Input: part model. Units: mm. Frame: model coordinates. A direction names the side the tool comes from. Give positions to 0.01 mm unless a question says otherwise; leave off trailing zeros. Loops run counter-clockwise (first coordinate to the right, second up) from the corner with the lowest first, then second, coordinate; pieces in that order, holes last.
from build123d import *

# Parameters (mm, degrees)
BOSS_EXTRUDE1_DEPTH     = 235
CUT_EXTRUDE1_DEPTH      = 252.322501977
CUT_EXTRUDE1_DEPTH_BACK = 252.322501977
SKETCH_1_R              = 16


with BuildPart() as part:
    # Sketch1 → Boss-Extrude1 (new, symmetric)
    with BuildSketch(Plane.XY):
        with BuildLine():
            Line((-53, -63), (53, -63))
            ThreePointArc((53, -63), (60.071067812, -60.071067812), (63, -53))
            Line((63, -53), (63, 53))
            ThreePointArc((63, 53), (60.071067812, 60.071067812), (53, 63))
            Line((53, 63), (-53, 63))
            ThreePointArc((-53, 63), (-60.071067812, 60.071067812), (-63, 53))
            Line((-63, 53), (-63, -53))
            ThreePointArc((-63, -53), (-60.071067812, -60.071067812), (-53, -63))
        make_face()
        with BuildLine():
            Line((-53, -58), (53, -58))
            ThreePointArc((53, -58), (56.535533906, -56.535533906), (58, -53))
            Line((58, -53), (58, 53))
            ThreePointArc((58, 53), (56.535533906, 56.535533906), (53, 58))
            Line((53, 58), (-53, 58))
            ThreePointArc((-53, 58), (-56.535533906, 56.535533906), (-58, 53))
            Line((-58, 53), (-58, -53))
            ThreePointArc((-58, -53), (-56.535533906, -56.535533906), (-53, -58))
        make_face(mode=Mode.SUBTRACT)
    extrude(amount=BOSS_EXTRUDE1_DEPTH, both=True)

    # 草图1 → Cut-Extrude1 (cut, two sides: drawn at the far end of the back side and taken through both)
    with BuildSketch(Plane(origin=(0, 0, 0), x_dir=(1, 0, 0), z_dir=(0, 1, 0)).offset(-CUT_EXTRUDE1_DEPTH_BACK)):
        with Locations(Location((0, 155, 0), (0, 0, 270))):
            Circle(SKETCH_1_R)
    extrude(amount=CUT_EXTRUDE1_DEPTH + CUT_EXTRUDE1_DEPTH_BACK, mode=Mode.SUBTRACT)


solid = part.part
(1) Cut plane C-C (x = -38.5). Return the cut outline in (y, z).
Values follow:
outline: (-63, -235) - (-58, -235) - (-58, 235) - (-63, 235) - close; (58, -235) - (63, -235) - (63, 235) - (58, 235) - close
(2) Cut plane B-B (z = 119). Return the cut outline in (x, y).
Values follow:
outline: (-63, -53) arc R10 ccw to (-53, -63) - (53, -63) arc R10 ccw to (63, -53) - (63, 53) arc R10 ccw to (53, 63) - (-53, 63) arc R10 ccw to (-63, 53) - close; hole (-58, -53) arc R5 ccw to (-53, -58) - (53, -58) arc R5 ccw to (58, -53) - (58, 53) arc R5 ccw to (53, 58) - (-53, 58) arc R5 ccw to (-58, 53) - close
(3) Cut plane A-A (x = 0). Return the cut outline in (y, z), and give its area (3 significant figures).
Values follow:
outline: (-63, -235) - (-58, -235) - (-58, -171) - (-63, -171) - close; (-63, -139) - (-58, -139) - (-58, 235) - (-63, 235) - close; (58, -235) - (63, -235) - (63, -171) - (58, -171) - close; (58, -139) - (63, -139) - (63, 235) - (58, 235) - close
area: 4,380 mm2
(4) Mould query, pull axis Z, two halves, no side actions, for faces 3 (the flat face through (0, 61, 235)), 4 (the cylindrical face through (-60.15, -59.99, 3.29)), 5 (the cylindrical face through (-14.195, -60.535, -147.617)). Classes: +Z half, -Z half, draft (parallel to the pull), parting line (faces both ways), or undercut.
Values follow:
face 3: +Z half
face 4: draft
face 5: undercut
(5) Ray query, probe 1 along Y at (x, z) = (47, 42.5); probe 2 along Z at (x, y) = (0, -61). Return the intervals inside material, ascending.
Values follow:
probe 1: y = -63 to -58, 58 to 63
probe 2: z = -235 to -171, -139 to 235
(6) Reachability of faces 1 (the flat face through (0, 61, -235)), 2 (the flat face through (58, -1, 3)) from +Z, -Z, +X, -X, +Y, -Y: full face, straight path, thin tool, end or side. Return the list, or none.
Values follow:
face 1: -Z, +X, -X, +Y, -Y
face 2: +Z, -Z
